Build history of the part. All positions in model axes, mm. A direction names the side the tool comes from. Coordinates: 2 decimals unless noted, no trailing zeros. Order: outer loops, then holes, each group sorted by start corner. A loop starts at its lowest first (then second) coordinate and runs counter-clockwise, first axis right, second up. Notation, with made-up numbers: (78.5, -22.5) - (107.5, -22.5) arc R25 ccw to (107.5, 13.5) - close; hole circle Ø10 at (-16.5, 49.25). An arc over 180 degrees is marked (long way). One line per item, written item: value.
from build123d import *
from build123d.topology import SkipClean

# Parameters (mm, degrees)
BASE_PLATE_SKETCH_140X105_W  = 105
BASE_PLATE_SKETCH_140X105_H  = 140
BASE_PLATE_DEPTH             = 12.5
HUB_BOSS_DEPTH               = 35
BORE_RELIEF_56_DEPTH         = 95.240384125
FILLER_START                 = -35
FILLER_BOSS_DEPTH            = 35
LUG_BOSS_DEPTH               = 25
SIDE_START                   = 20
SIDE_EAR_SKETCH_R            = 5
SIDE_EAR_DEPTH               = 15
MOUNTING_HOLES_SKETCH_10_R   = 5
MOUNTING_HOLES_SKETCH_10_R_2 = 20
MOUNTING_HOLES_10_DEPTH      = 110.001146783


with BuildPart() as part:
    # Base Plate Sketch 140x105 → Base Plate (new, symmetric)
    with BuildSketch(Plane(origin=(0, 0, 0), x_dir=(1, 0, 0), z_dir=(0, 1, 0))):
        Rectangle(BASE_PLATE_SKETCH_140X105_W, BASE_PLATE_SKETCH_140X105_H)
    extrude(amount=BASE_PLATE_DEPTH, both=True)

    # Hub Boss Sketch → Hub Boss (add)
    with BuildSketch(Plane(origin=(0, 12.5, 0), x_dir=(1, 0, 0), z_dir=(0, 1, 0))):
        with BuildLine():
            Line((-17.5, 70), (-35, 70))
            Line((-35, 70), (-35, 14))
            Line((-35, 14), (-35, -35))
            ThreePointArc((-35, -35), (-24.748737337, -59.748737346), (1.3e-08, -70))
            ThreePointArc((1.3e-08, -70), (24.748737346, -59.748737337), (35, -35))
            Line((35, -35), (35, 14))
            Line((35, 14), (35, 70))
            Line((35, 70), (17.5, 70))
            Line((17.5, 70), (-17.5, 70))
        make_face()
    extrude(amount=-HUB_BOSS_DEPTH)

    # Bore Relief Sketch _56 → Bore Relief _56 (cut, through all)
    with SkipClean():  # the faces are left unmerged after this step: merging them gives an invalid solid
        with BuildSketch(Plane(origin=(0, 12.5, 0), x_dir=(1, 0, 0), z_dir=(0, 1, 0))):
            with BuildLine():
                Line((-52.5, -70), (6e-09, -70))
                ThreePointArc((6e-09, -70), (-24.748737339, -59.748737344), (-35, -35))
                ThreePointArc((-35, -35), (-32.267021942, -21.441264992), (-24.494897428, -10))
                ThreePointArc((-24.494897428, -10), (-21.331375002, 5.291502622), (-34.292856399, 14))
                Line((-34.292856399, 14), (-52.5, 14))
                Line((-52.5, 14), (-52.5, -70))
            make_face()
            with BuildLine():
                Line((52.5, -70), (52.5, 14))
                Line((52.5, 14), (34.292856399, 14))
                ThreePointArc((34.292856399, 14), (21.331375002, 5.291502622), (24.494897428, -10))
                ThreePointArc((24.494897428, -10), (32.267021942, -21.441264992), (35, -35))
                ThreePointArc((35, -35), (24.748737344, -59.748737339), (6e-09, -70))
                Line((6e-09, -70), (52.5, -70))
            make_face()
        extrude(amount=-BORE_RELIEF_56_DEPTH, mode=Mode.SUBTRACT)

    # Filler Boss Sketch → Filler Boss (add)
    with SkipClean():  # the faces are left unmerged after this step: merging them gives an invalid solid
        with BuildSketch(Plane.XZ.offset(22.5).offset(FILLER_START)):
            with BuildLine():
                Line((-34.292856399, -14), (-34.292856399, 28))
                ThreePointArc((-34.292856399, 28), (-30.740852298, 18.266799469), (-24.494897428, 10))
                ThreePointArc((-24.494897428, 10), (-21.331375002, -5.291502622), (-34.292856399, -14))
            make_face()
            with BuildLine():
                Line((34.292856399, -14), (34.292856399, 28))
                ThreePointArc((34.292856399, 28), (30.740852298, 18.266799469), (24.494897428, 10))
                ThreePointArc((24.494897428, 10), (21.331375002, -5.291502622), (34.292856399, -14))
            make_face()
        extrude(amount=FILLER_BOSS_DEPTH)

    # Lug Boss Sketch → Lug Boss (add)
    with SkipClean():  # the faces are left unmerged after this step: merging them gives an invalid solid
        with BuildSketch(Plane(origin=(0, 12.5, 0), x_dir=(1, 0, 0), z_dir=(0, 1, 0))):
            with BuildLine():
                Line((48.292856399, 14), (34.292856399, 14))
                Line((34.292856399, 14), (34.292856399, 0))
                ThreePointArc((34.292856399, 0), (38.393361462, 9.899494937), (48.292856399, 14))
            make_face()
            with BuildLine():
                Line((-34.292856399, 0), (-34.292856399, 14))
                Line((-34.292856399, 14), (-48.292856399, 14))
                ThreePointArc((-48.292856399, 14), (-38.393361462, 9.899494937), (-34.292856399, 0))
            make_face()
        extrude(amount=-LUG_BOSS_DEPTH)

    # Side Ear Sketch → Side Ear (add)
    with SkipClean():  # the faces are left unmerged after this step: merging them gives an invalid solid
        with BuildSketch(Plane(origin=(0, 0, 0), x_dir=(0, 0, -1), z_dir=(1, 0, 0)).offset(SIDE_START)):
            with BuildLine():
                Line((70, -37.5), (70, -22.5))
                Line((70, -22.5), (14, -22.5))
                Line((14, -22.5), (42.254134702, -45.408408045))
                ThreePointArc((42.254134702, -45.408408045), (47.707062344, -50.607748103), (55, -52.5))
                ThreePointArc((55, -52.5), (65.606601718, -48.106601718), (70, -37.5))
            make_face()
            with Locations((55, -37.5)):
                Circle(SIDE_EAR_SKETCH_R, mode=Mode.SUBTRACT)
        side_ear = extrude(amount=SIDE_EAR_DEPTH)

    # Side Ear Mirror: Side Ear across plane
    with SkipClean():  # the faces are left unmerged after this step: merging them gives an invalid solid
        add(side_ear.mirror(Plane(origin=(0, 0, 0), x_dir=(0, 0, 1), z_dir=(1, 0, 0))))

    # Mounting Holes Sketch _10 → Mounting Holes _10 (cut, through all)
    with SkipClean():  # the faces are left unmerged after this step: merging them gives an invalid solid
        with BuildSketch(Plane(origin=(0, 12.5, 0), x_dir=(1, 0, 0), z_dir=(0, 1, 0))):
            with Locations(Location((-42.5, 47, 0), (0, 0, 270))):
                Circle(MOUNTING_HOLES_SKETCH_10_R)
            with Locations(Location((42.5, 47, 0), (0, 0, 270))):
                Circle(MOUNTING_HOLES_SKETCH_10_R)
            with Locations(Location((0, -35, 0), (0, 0, 270))):
                Circle(MOUNTING_HOLES_SKETCH_10_R_2)
        extrude(amount=-MOUNTING_HOLES_10_DEPTH, mode=Mode.SUBTRACT)


solid = part.part
1. Band-saw the part on C-C, the plane y = -36. Give the cut face in (x, z), and give its area (3 significant figures).
Values found:
outline: (-35, -70) - (-20, -70) - (-20, -59.77) - (-35, -59.77) - close; (-35, -50.23) - (-20, -50.23) - (-20, -30.65) - (-35, -30.65) - close; (20, -70) - (35, -70) - (35, -59.77) - (20, -59.77) - close; (20, -50.23) - (35, -50.23) - (35, -30.65) - (20, -30.65) - close
area: 894 mm2
2. Probe line 1 along X through (y, z) = (-6.5, -47); line 2 along Y through (x, z) = (-27, -55); line 3 along X through (y, z) = (6, -43.5). List the from-to ranges inside material, lowest first.
Values found:
line 1: x = -52.5 to -47.5, -37.5 to 37.5, 47.5 to 52.5
line 2: y = -52.5 to -42.5, -32.5 to 12.5
line 3: x = -52.5 to -46.07, -38.93 to 38.93, 46.07 to 52.5
3. Two-plate mould, pull along Y, no slides. Class faces 1 (the face through (-39.121, 0.175, -50.685)), 2 (the face through (-27.395, -34.121, -51.315)), 3 (the face through (-27.395, -33.794, -27.929)): pulls with the +Y half, pulls with the -Y half, needs draft (parallel to the pull), parting line crosses it, or undercut.
Values found:
face 1: needs draft
face 2: undercut
face 3: pulls with the -Y half
4. Band-saw the part on B-B, the plane z = 51. Give the cut face in (x, y), and give its area (3 significant figures).
Values found:
outline: (-31.13, -22.5) - (-12, -22.5) - (-12, 12.5) - (-31.13, 12.5) - close; (12, -22.5) - (31.13, -22.5) - (31.13, 12.5) - (12, 12.5) - close
area: 1,340 mm2
5. 3-axis set-ups, long thin cutter, end or side, ignore diameter. For faces 4 (the face through (50, 0, -14)), 5 (the face through (-50, 0, -14)), 6 (the face through (20, -34, -48)), 7 (the face through (34.293, -5, 11)): which of +Z, -Z, +X, -X, +Y, -Y reach the whole face in a straight line?
Values found:
face 4: +Z, +X, +Y, -Y
face 5: +Z, -X, +Y, -Y
face 6: +Z, -Z, -Y
face 7: +X, -Y
6. Band-saw the part on A-A, the plane x = -6.5. Give the cut face in (y, z), and give its area (3 significant figures).
Values found:
outline: (-22.5, -70) - (12.5, -70) - (12.5, 16.09) - (-22.5, 16.09) - close; (-22.5, 53.91) - (12.5, 53.91) - (12.5, 69.39) - (-22.5, 69.39) - close
area: 3,550 mm2
7. Band-saw the part on D-D, the plane y = -7. Give the cut face in (x, z).
Values found:
outline: (-52.5, -70) - (52.5, -70) - (52.5, -14) - (48.29, -14) arc R14 cw to (34.29, 0) - (34.29, 28) arc R35 ccw (long way) to (-34.29, 28) - (-34.29, 0) arc R14 cw to (-48.29, -14) - (-52.5, -14) - close; hole circle Ø10 at (-42.5, -47); hole circle Ø40 at (0, 35); hole circle Ø10 at (42.5, -47)
8. Flat gauge pins, fed straight in: P1, Ø11, axis at x = 27.5, z = 10, coming from the -Y side; P2, Ø9, axis at x = -45.5, z = -43.5, coming from the -Y side; P3, Ø5, axis at y = -18, z = -55, coming from the +X side. Where does each tip first touch, or does it go through?
Values found:
P1: stops at y = -22.5
P2: stops at y = -12.5
P3: stops at x = 35
